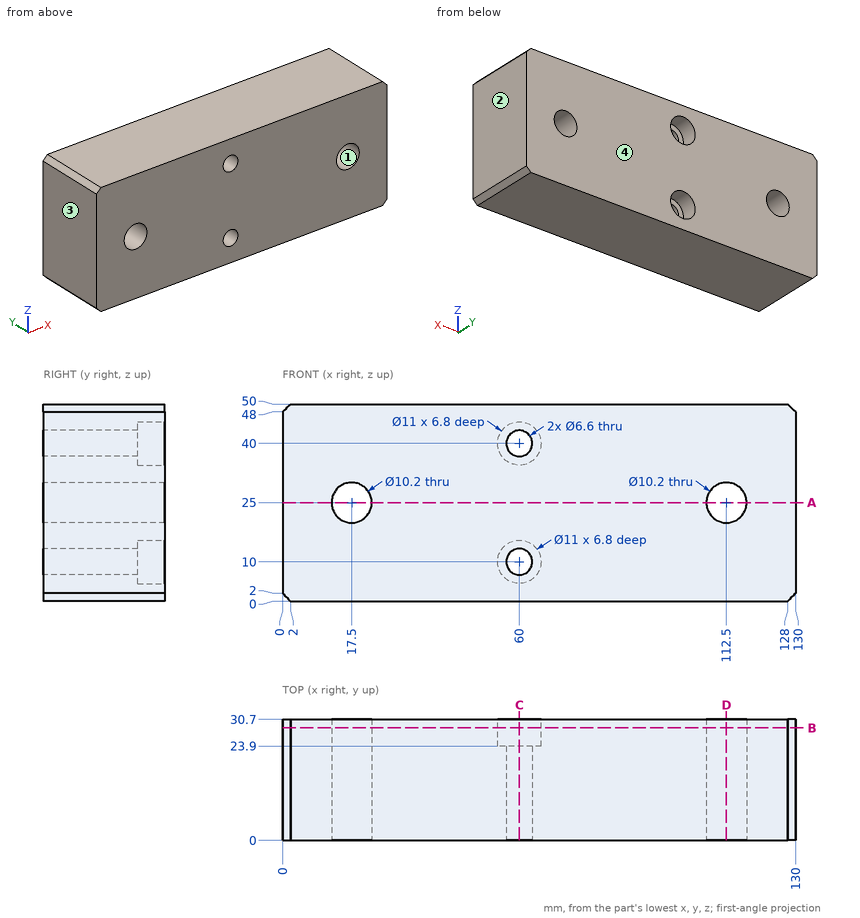
Here's the drawing with two shaded views (mm, measured from the low corner). I have some questions. Coordinates: 2 decimals unless noted, no trailing zeros. Write each loop counter-clockwise with the first axis right and the second up, starting at its lowest first coordinate (ties: lowest second). Pieces come first, ordered by that corner, then holes. Notation, with made-up numbers: M 25,29 L 42,29 A17 cw 42,37 Z; hole C -22,67.5 d10. An arc over 180 degrees is marked long. Write item = value, one per line. Start each with the question number.
Q1. Thinking about a two-plate mould opening in X: for the marked faces 1, 2, 3 and 4, which applies, released by +X, released by -X, zero draft, split by the parting line, or undercut?
Q2. If we section it at B-B, the plane y = 28.5: Write out the boundary of the cut face in (x, z), then the cut area to 3 significant figures.
Q3. If we section it at C-C, the plane x = 60: Write out the boundary of the cut face in (y, z), then the cut area to 3 significant figures.
Q4. I'm going to push flat-ended pins straight in: pin 1 (5.5 mm diameter, centred on x = 60, z = 8, fed in from +Y); pin 2 (6 mm diameter, centred on x = 60, z = 40, fed in from -Y). Where does each tip first touch, or does it pass through?
Q5. If we section it at D-D, the plane x = 112.5: Write out the boundary of the cut face in (y, z).
Q6. If I drill on L1, parallel to Z at x = 60, y = 14; L2, parallel to Z at x = 60, y = 29.5; L3, parallel to Z at x = 18, y = 14, over which ranges is the centre line in solid material (lowest first)? Write a range as [from, to].
Q7. If we section it at A-A, the plane z = 25: Write out the boundary of the cut face in (x, y), then the cut area to 3 significant figures.
Check sheet entries:
q1.face_1 = undercut
q1.face_2 = released by +X
q1.face_3 = released by -X
q1.face_4 = zero draft
q2.outline = M 0,2 L 2,0 L 128,0 L 130,2 L 130,48 L 128,50 L 2,50 L 0,48 Z; hole C 17.5,25 d10.2; hole C 60,10 d11; hole C 60,40 d11; hole C 112.5,25 d10.2
q2.area = 6,140 mm²
q3.outline = M 0,0 L 30.7,0 L 30.7,4.5 L 23.9,4.5 L 23.9,6.7 L 0,6.7 Z; M 0,13.3 L 23.9,13.3 L 23.9,15.5 L 30.7,15.5 L 30.7,34.5 L 23.9,34.5 L 23.9,36.7 L 0,36.7 Z; M 0,43.3 L 23.9,43.3 L 23.9,45.5 L 30.7,45.5 L 30.7,50 L 0,50 Z
q3.area = 1,070 mm²
q4.pin_1 = 23.9
q4.pin_2 = through
q5.outline = M 0,0 L 30.7,0 L 30.7,19.9 L 0,19.9 Z; M 0,30.1 L 30.7,30.1 L 30.7,50 L 0,50 Z
q6.L1 = [0, 6.7], [13.3, 36.7], [43.3, 50]
q6.L2 = [0, 4.5], [15.5, 34.5], [45.5, 50]
q6.L3 = [0, 19.92], [30.08, 50]
q7.outline = M 0,0 L 12.4,0 L 12.4,30.7 L 0,30.7 Z; M 22.6,0 L 107.4,0 L 107.4,30.7 L 22.6,30.7 Z; M 117.6,0 L 130,0 L 130,30.7 L 117.6,30.7 Z
q7.area = 3,360 mm²
